Geometry check sheet. Reference: drawing and pictorial views, mm from the part's lowest x, y, z. A direction names the side the tool comes from. Round coordinates to 2 decimals unless told otherwise and drop trailing zeros. Order: outer loops, then holes, each group sorted by start corner. A loop starts at its lowest first (then second) coordinate and runs counter-clockwise, first axis right, second up.
(1) Thickness scan on probe 1 along X at (y, z) = (4.5, 20); probe 2 along Z at (x, y) = (8, 7.25); probe 3 along Y at (x, z) = (50, 16.5). Record the ranges inside material, lowest first.
(2) Sectioned sample at D-D, the plane x = 92. Enter the section's corners in (y, z), and give its area (3 significant figures).
(3) Sectioned sample at B-B, the plane x = 50. Enter the section's corners in (y, z), and give its area (3 significant figures).
(4) Tool access check on the marked faces 1, 2, 3, 4 and 5. Record the directions out of +Z, -Z, +X, -X, +Y, -Y that give a thin tool (end or side, any length) a straight path to the whole face; none if there is none.
(5) Sectioned sample at C-C, the plane y = 6.5. Enter the section's corners in (x, z).
(6) Sectioned sample at A-A, the plane z = 20. Enter the section's corners in (x, y), and give its area (3 significant figures).
(7) Depth check by flat-ended pin: pin 1 (11 mm diameter, centred on x = 47.5, z = 35, fed in from +Y); pin 2 (1 mm diameter, centred on x = 13, z = 23, fed in from +Y); pin 3 (8 mm diameter, centred on x = 75, y = 59.5, fed in from +Z). Enter the tip coordinate at first touch or a pass-through.
(8) Mould release check, pull along X, two halves, no side actions. Record for the marked faces 6, 7 and 8: released by +X, released by -X, zero draft, split by the parting line, or undercut.
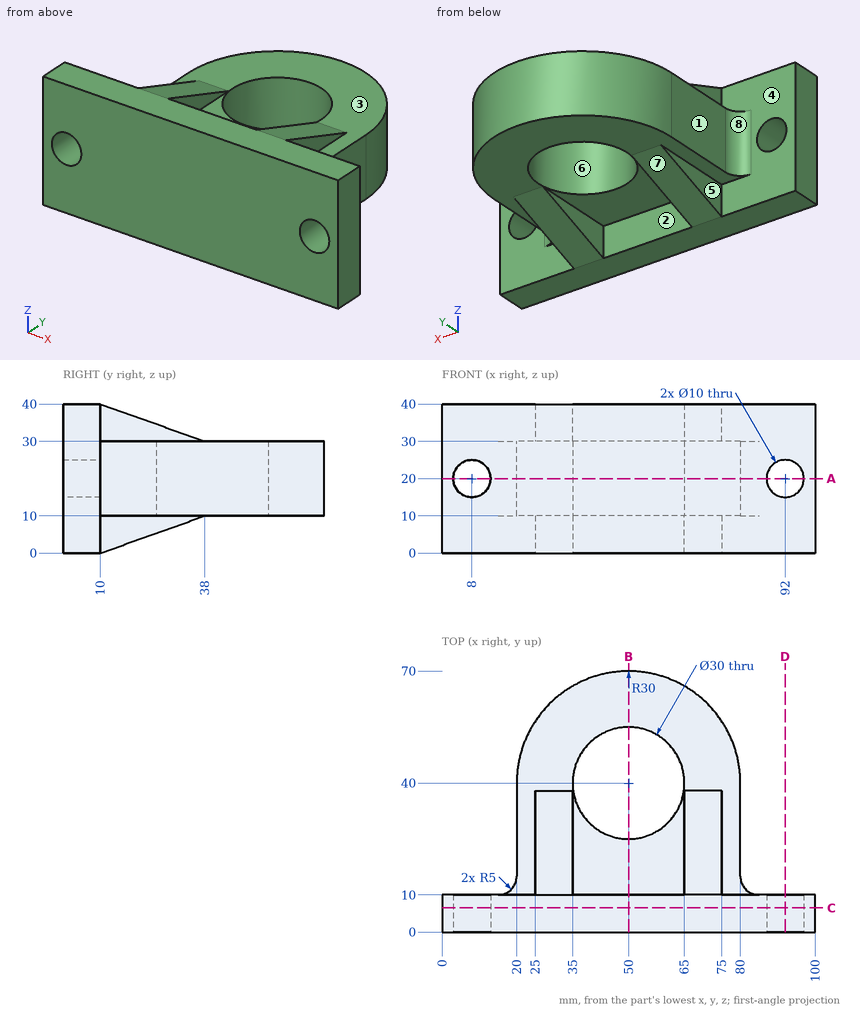
Derived:
1. probe 1: x = 0 to 3, 13 to 87, 97 to 100
1. probe 2: z = 0 to 15, 25 to 40
1. probe 3: y = 0 to 25, 55 to 70
2. outline: (0, 0) - (10, 0) - (10, 15) - (0, 15) - close; (0, 25) - (10, 25) - (10, 40) - (0, 40) - close
2. area: 300 mm2
3. outline: (0, 0) - (10, 0) - (10, 10) - (25, 10) - (25, 30) - (10, 30) - (10, 40) - (0, 40) - close; (55, 10) - (70, 10) - (70, 30) - (55, 30) - close
3. area: 1,000 mm2
4. face 1: +Z, -Z, -X, +Y
4. face 2: -Z, +Y
4. face 3: +Z, +Y
4. face 4: -X, +Y
4. face 5: -Z, -X, +Y
5. outline: (0, 0) - (100, 0) - (100, 40) - (0, 40) - close; hole circle Ø10 at (8, 20); hole circle Ø10 at (92, 20)
6. outline: (0, 0) - (3, 0) - (3, 10) - (0, 10) - close; (13, 0) - (87, 0) - (87, 10) - (85, 10) arc R5 cw to (80, 15) - (80, 40) arc R30 ccw to (20, 40) - (20, 15) arc R5 cw to (15, 10) - (13, 10) - close; (97, 0) - (100, 0) - (100, 10) - (97, 10) - close; hole circle Ø30 at (50, 40)
6. area: 3,320 mm2
7. pin 1: stops at y = 70
7. pin 2: stops at y = 10
7. pin 3: stops at z = 30
8. face 6: undercut
8. face 7: zero draft
8. face 8: released by -X
